from build123d import *

# Parameters (mm, degrees)
SWEEP_THIN_PART_1_PROFILE_R   = 30.15
SWEEP_THIN_PART_1_PROFILE_R_2 = 25
SWEEP_THIN_PART_2_PROFILE_R   = 30.15
SWEEP_THIN_PART_2_PROFILE_R_2 = 25
SKETCH15_R                    = 25
CUT_EXTRUDE1_DEPTH            = 177.264070494
SKETCH18_R                    = 25
CUT_EXTRUDE2_DEPTH            = 85


with BuildPart() as part:
    # Sweep-thin part 1: sweep along a path in Sketch1
    with BuildLine(Plane.XY) as sweep_thin_part_1_path:
        Line((-76, 0), (76, 0))
    # Sweep-thin part 1 profile (on start of the path) → Sweep-thin part 1 (sweep)
    with BuildSketch(Plane.YZ.offset(-76)):
        Circle(SWEEP_THIN_PART_1_PROFILE_R)
        Circle(SWEEP_THIN_PART_1_PROFILE_R_2, mode=Mode.SUBTRACT)
    sweep(path=sweep_thin_part_1_path.line)

    # Sweep-thin part 2: sweep along a path in Sketch8
    with BuildLine(Plane.XY) as sweep_thin_part_2_path:
        Line((0, 0), (0, -84))
    # Sweep-thin part 2 profile (on start of the path) → Sweep-thin part 2 (sweep)
    with BuildSketch(Plane(origin=(0, 0, 0), x_dir=(-1, 0, 0), z_dir=(0, -1, 0))):
        Circle(SWEEP_THIN_PART_2_PROFILE_R)
        Circle(SWEEP_THIN_PART_2_PROFILE_R_2, mode=Mode.SUBTRACT)
    sweep(path=sweep_thin_part_2_path.line)

    # Sketch15 → Cut-Extrude1 (cut, through all)
    with BuildSketch(Plane.ZY.offset(76)):
        with Locations(Location((0, 0, 0), (0, 0, 90))):
            Circle(SKETCH15_R)
    extrude(amount=-CUT_EXTRUDE1_DEPTH, mode=Mode.SUBTRACT)

    # Sketch18 → Cut-Extrude2 (cut)
    with BuildSketch(Plane.XZ.offset(84)):
        Circle(SKETCH18_R)
    extrude(amount=-CUT_EXTRUDE2_DEPTH, mode=Mode.SUBTRACT)


solid = part.part
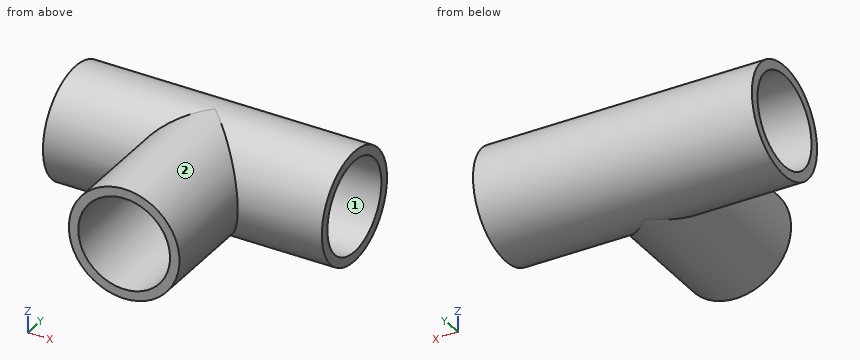
Geometry: final body of the model. Coordinates: model frame, mm. Face numbers are marked on the shaded views. Give positions to 0.01 mm unless a question says otherwise; leave off trailing zeros. Write each loop counter-clockwise with the first axis right and the second up, starting at its lowest first coordinate (ties: lowest second). Pieces come first, ordered by that corner, then holes. Notation, with made-up numbers: (-13.75, 76) -> (-7.75, 76) arc R20 cw to (-7.75, 108) -> close; hole circle Ø5 at (-6.5, 56). An arc over 180 degrees is marked (long way). Answer as a JSON object with one key per item and string values.
1. Cut plane D-D on y = -3.5. Output: boundary loops of the cut face in (x, z).
Ans:
{"outline": "(-76, -29.95) -> (-3.5, -29.95) arc R30.15 ccw to (3.5, -29.95) -> (76, -29.95) -> (76, -24.75) -> (3.5, -24.75) arc R25 cw to (-3.5, -24.75) -> (-76, -24.75) -> close; (-76, 24.75) -> (-3.5, 24.75) arc R25 cw to (3.5, 24.75) -> (76, 24.75) -> (76, 29.95) -> (3.5, 29.95) arc R30.15 ccw to (-3.5, 29.95) -> (-76, 29.95) -> close"}
2. Mould query, pull axis Z, two halves, no side actions, for the marked faces 1 and 2. Classes: pulls with the +Z half, pulls with the -Z half, needs draft (parallel to the pull), parting line crosses it, or undercut.
Ans:
{"face 1": "undercut", "face 2": "parting line crosses it"}
3. Ray query, probe 1 along Z at (x, y) = (0, -54); probe 2 along Z at (x, y) = (17.5, -43); probe 3 along X at (y, z) = (-66, -16). Return the intervals inside material, ascending. Write a range as from..to.
Ans:
{"probe 1": "z = -30.15..-25, 25..30.15", "probe 2": "z = -24.55..-17.85, 17.85..24.55", "probe 3": "x = -25.55..-19.21, 19.21..25.55"}
4. Cut plane B-B on z = -19. Output: boundary loops of the cut face in (x, y).
Ans:
{"outline": "(-76, -23.41) -> (-23.41, -23.41) -> (-23.41, -84) -> (-16.25, -84) -> (-16.25, -16.25) -> (-76, -16.25) -> close; (-76, 16.25) -> (76, 16.25) -> (76, 23.41) -> (-76, 23.41) -> close; (16.25, -84) -> (23.41, -84) -> (23.41, -23.41) -> (76, -23.41) -> (76, -16.25) -> (16.25, -16.25) -> close"}
5. Contact query for flat-ended pins moving along their axis: pin 1 (3 mm diameter, centred on x = -27.5, z = 18, fed in from +Y); pin 2 (8 mm diameter, centred on x = -49.5, z = 3.5, fed in from +Y); pin 3 (2 mm diameter, centred on y = -57, z = -6.5, fed in from +X); pin 4 (2 mm diameter, centred on x = -2.5, z = -17.5, fed in from -Y). Output: stop coordinate, or through.
Ans:
{"pin 1": "stops at y = 25.23", "pin 2": "stops at y = 30.15", "pin 3": "stops at x = 29.64", "pin 4": "stops at y = 16.82"}
6. Cut plane A-A on x = -55. Output: boundary loops of the cut face in (y, z), and give its area (3 significant figures).
Ans:
{"outline": "circle Ø60.3 at (0, 0); hole circle Ø50 at (0, 0)", "area": "892 mm^2"}
